from build123d import *

# Parameters (mm, degrees)
SKETCH1_W           = 15
SKETCH1_H           = 120
BOSS_EXTRUDE1_DEPTH = 76
SKETCH2_R           = 5
CUT_EXTRUDE2_DEPTH  = 98.119771417


with BuildPart() as part:
    # Sketch1 → Boss-Extrude1 (new body)
    with BuildSketch(Plane.XY):
        Rectangle(SKETCH1_W, SKETCH1_H)
    extrude(amount=BOSS_EXTRUDE1_DEPTH)

    # Sketch2 → Cut-Extrude2 (cut, through all)
    with BuildSketch(Plane.XY.offset(76)):
        with Locations((0, 11)):
            Circle(SKETCH2_R)
    extrude(amount=-CUT_EXTRUDE2_DEPTH, mode=Mode.SUBTRACT)


solid = part.part
Input: part model. Units: mm. Frame: model coordinates. Give positions to 0.01 mm unless a question says otherwise; leave off trailing zeros. Write each loop counter-clockwise with the first axis right and the second up, starting at its lowest first coordinate (ties: lowest second). Pieces come first, ordered by that corner, then holes.
Q1. Material intervals for probe 1 along Y at (x, z) = (0.5, 22); probe 2 along Y at (x, z) = (4, 33); probe 3 along X at (y, z) = (12, 10), sorted ascending.
Q2. Section C-C, the plane z = 54. Output: boundary loops of the cut face in (x, y), plus the area to 3 significant figures.
Q3. Pull-direction query (X, two-part tool) for faces 1 (the face through (0, 60, 37)), 2 (the face through (7.5, -1, 37)), 3 (the face through (-0.651, 15.957, 38.532)); classes: pulls with the +X half, pulls with the -X half, needs draft (parallel to the pull), parting line crosses it, or undercut.
Q4. Section A-A, the plane x = 0. Output: boundary loops of the cut face in (y, z), plus the area to 3 significant figures.
Q5. Section B-B, the plane y = 11. Output: boundary loops of the cut face in (x, z), plus the area to 3 significant figures.
Filled in:
1. probe 1: y = -60 to 6.03, 15.97 to 60
1. probe 2: y = -60 to 8, 14 to 60
1. probe 3: x = -7.5 to -4.9, 4.9 to 7.5
2. outline: (-7.5, -60) - (7.5, -60) - (7.5, 60) - (-7.5, 60) - close; hole circle Ø10 at (0, 11)
2. area: 1,720 mm2
3. face 1: needs draft
3. face 2: pulls with the +X half
3. face 3: undercut
4. outline: (-60, 0) - (6, 0) - (6, 76) - (-60, 76) - close; (16, 0) - (60, 0) - (60, 76) - (16, 76) - close
4. area: 8,360 mm2
5. outline: (-7.5, 0) - (-5, 0) - (-5, 76) - (-7.5, 76) - close; (5, 0) - (7.5, 0) - (7.5, 76) - (5, 76) - close
5. area: 380 mm2
